from build123d import *

# Parameters (mm, degrees)
SKETCH_1_R                   = 58
EXTRUDE_1_DEPTH              = 3
SKETCH_2_R                   = 47.25
SKETCH_2_R_2                 = 42.25
EXTRUDE_2_DEPTH              = 30
CHAMFER_1_SIZE               = 0.5
HOLE_WIZARD_M4_1_D           = 4.2
HOLE_WIZARD_M4_1_DEPTH       = 10.1
HOLE_WIZARD_M4_1_CSINK_D     = 8
HOLE_WIZARD_M4_1_CSINK_ANGLE = 90
HOLE_WIZARD_M4_1_TIP         = 1.2618073
HOLE_WIZARD_M3_2_D           = 2.5
HOLE_WIZARD_M3_2_DEPTH       = 7.5
HOLE_WIZARD_M3_2_TIP         = 0.751075774
SKETCH_32_R                  = 4.1
CUT_EXTRUDE_12_DEPTH         = 1.4


with BuildPart() as part:
    # 草图1 → 凸台-拉伸1 (new body)
    with BuildSketch(Plane.XY):
        Circle(SKETCH_1_R)
    extrude(amount=EXTRUDE_1_DEPTH)

    # 草图2 → 凸台-拉伸2 (add)
    with BuildSketch(Plane.XY.offset(3)):
        Circle(SKETCH_2_R)
        Circle(SKETCH_2_R_2, mode=Mode.SUBTRACT)
    extrude(amount=EXTRUDE_2_DEPTH)

    # 倒角1
    chamfer_1_edges = [part.edges().sort_by_distance(p)[0] for p in [
        (-58, 0, 0),
    ]]
    chamfer(chamfer_1_edges, length=CHAMFER_1_SIZE)

    # M4 六角凹锥坑螺钉的锥形沉头孔1
    with Locations(Plane(origin=(0, 0, 0), x_dir=(-1, 0, 0), z_dir=(0, 0, -1))):
        with Locations((0, 53), (53, 0), (0, -53), (-53, 0)):
            CounterSinkHole(HOLE_WIZARD_M4_1_D / 2, HOLE_WIZARD_M4_1_CSINK_D / 2, depth=HOLE_WIZARD_M4_1_DEPTH, counter_sink_angle=HOLE_WIZARD_M4_1_CSINK_ANGLE)
            with Locations((0, 0, -(HOLE_WIZARD_M4_1_DEPTH + HOLE_WIZARD_M4_1_TIP / 2))):  # 118° drill point
                Cone(0, HOLE_WIZARD_M4_1_D / 2, HOLE_WIZARD_M4_1_TIP, mode=Mode.SUBTRACT)

    # M3 螺纹孔2
    with Locations(Plane.XY.offset(33)):
        with Locations((0, 44.5), (44.5, 0), (0, -44.5), (-44.5, 0), (0, 0)):
            Hole(HOLE_WIZARD_M3_2_D / 2, depth=HOLE_WIZARD_M3_2_DEPTH)
            with Locations((0, 0, -(HOLE_WIZARD_M3_2_DEPTH + HOLE_WIZARD_M3_2_TIP / 2))):  # 118° drill point
                Cone(0, HOLE_WIZARD_M3_2_D / 2, HOLE_WIZARD_M3_2_TIP, mode=Mode.SUBTRACT)

    # 草图32 → 切除-拉伸12 (cut)
    with BuildSketch(Plane.XY.offset(3)):
        with Locations((37.476659403, -37.476659403)):
            Circle(SKETCH_32_R)
        with Locations(Location((37.476659403, 37.476659403, 0), (0, 0, 180))):
            Circle(SKETCH_32_R)
        with Locations((-37.476659403, 37.476659403)):
            Circle(SKETCH_32_R)
        with Locations(Location((-37.476659403, -37.476659403, 0), (0, 0, 180))):
            Circle(SKETCH_32_R)
    extrude(amount=-CUT_EXTRUDE_12_DEPTH, mode=Mode.SUBTRACT)


solid = part.part
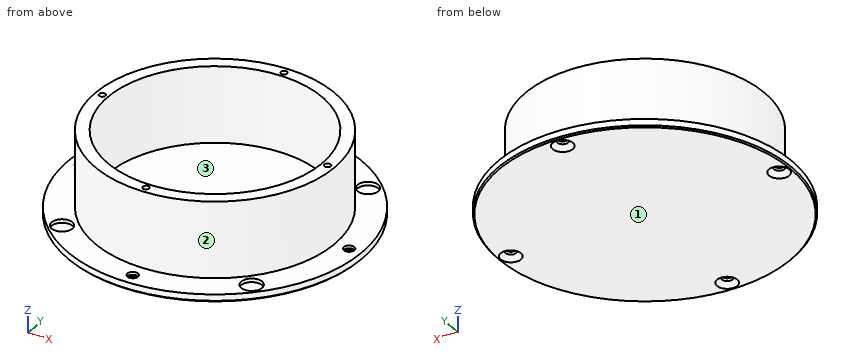
Geometry: final body of the model. Coordinates: model frame, mm. Face numbers are marked on the shaded views. Round coordinates to 2 decimals unless told otherwise and drop trailing zeros. Order: outer loops, then holes, each group sorted by start corner. A loop starts at its lowest first (then second) coordinate and runs counter-clockwise, first axis right, second up.
Q1. Section A-A, the plane z = 29. Output: boundary loops of the cut face in (x, y).
Result sheet:
outline: circle Ø94.5 at (0, 0); hole circle Ø2.5 at (-44.5, 0); hole circle Ø84.5 at (0, 0); hole circle Ø2.5 at (0, -44.5); hole circle Ø2.5 at (0, 44.5); hole circle Ø2.5 at (44.5, 0)
Q2. Material intervals for probe 1 along Y at (x, z) = (0, 27); probe 2 along Y at (x, z) = (0, 2.75); probe 3 along Z at (x, y) = (-31, 0.5), sorted ascending.
Result sheet:
probe 1: y = -47.25 to -45.75, -43.25 to -42.25, 42.25 to 43.25, 45.75 to 47.25
probe 2: y = -58 to -55.1, -50.9 to 50.9, 55.1 to 58
probe 3: z = 0 to 3
Q3. Section B-B, the plane z = 11. Output: boundary loops of the cut face in (x, y), and give its area (3 significant figures).
Result sheet:
outline: circle Ø94.5 at (0, 0); hole circle Ø84.5 at (0, 0)
area: 1,410 mm2
Q4. Mould query, pull axis X, two halves, no side actions, for the marked faces 1, 2 and 3. Classes: released by +X, released by -X, zero draft, split by the parting line, or undercut.
Result sheet:
face 1: zero draft
face 2: split by the parting line
face 3: undercut
Q5. Pin query (flat end, axial travel): pin 1 (1.5 mm diameter, centred on x = 30.5, z = 7.5, fed in from -Y); pin 2 (4 mm diameter, centred on x = -19, z = 23, fed in from +Y); pin 3 (5 mm diameter, centred on y = -42, z = 20.5, fed in from -X). Return the tip coordinate at first contact, or that it passes through.
Result sheet:
pin 1: stops at y = -36.71
pin 2: stops at y = 44.09
pin 3: stops at x = -25.93
